```python
from build123d import *

# Parameters (mm, degrees)
SKETCH_1_4_R        = 75
BOSS_EXTRUDE1_DEPTH = 18
SKETCH_1_3_R        = 50
BOSS_EXTRUDE2_DEPTH = 210
BOSS_EXTRUDE3_START = -228
SKETCH_1_4_2_R      = 75
BOSS_EXTRUDE3_DEPTH = 18


with BuildPart() as part:
    # Sketch 1_4 → Boss-Extrude1 (new body)
    with BuildSketch(Plane(origin=(0, 0, 0), x_dir=(0, 0, -1), z_dir=(1, 0, 0))):
        Circle(SKETCH_1_4_R)
    extrude(amount=BOSS_EXTRUDE1_DEPTH)

    # 草图1<3> → Boss-Extrude2 (add)
    with BuildSketch(Plane(origin=(0, 0, 0), x_dir=(0, 0, -1), z_dir=(1, 0, 0))):
        Circle(SKETCH_1_3_R)
    extrude(amount=-BOSS_EXTRUDE2_DEPTH)

    # Sketch 1_4 2 → Boss-Extrude3 (add)
    with BuildSketch(Plane(origin=(0, 0, 0), x_dir=(0, 0, -1), z_dir=(1, 0, 0)).offset(BOSS_EXTRUDE3_START)):
        Circle(SKETCH_1_4_2_R)
    extrude(amount=BOSS_EXTRUDE3_DEPTH)


solid = part.part
```
Here's how the part is built. I have some questions about the finished solid (model axes, mm). A direction names the side the tool comes from. Coordinates: 2 decimals unless noted, no trailing zeros. Order: outer loops, then holes, each group sorted by start corner. A loop starts at its lowest first (then second) coordinate and runs counter-clockwise, first axis right, second up. Notation, with made-up numbers: (-32, -11.75) - (-19, -11.75) arc R20 ccw to (-19, 21.25) - close; hole circle Ø10 at (-1, 51). An arc over 180 degrees is marked (long way). One line per question, with ' | ' between items.
(1) Will these pins go through, and if not, where does the flat tip stop? pin 1 (10 mm diameter, centred on x = -96, z = 37, fed in from +Y); pin 2 (12 mm diameter, centred on x = -123, y = 32, fed in from +Z); pin 3 (10 mm diameter, centred on x = -163, z = 20.5, fed in from +Y).
Report:
pin 1: stops at y = 38.42 | pin 2: stops at z = 42.71 | pin 3: stops at y = 47.54
(2) If we mould it in two halves opening along X, with no side actions, what happens to faces 1 (the flat face through (18, 1, 1)), 2 (the flat face through (-228, 1, 1)), 3 (the cylindrical face through (8.874, 74.362, 9.764)), 4 (the flat face through (-210, -16, -49))? For each: pulls with the +X half, pulls with the -X half, needs draft (parallel to the pull), parting line crosses it, or undercut.
Report:
face 1: pulls with the +X half | face 2: pulls with the -X half | face 3: needs draft | face 4: undercut
(3) If I drill on L1, parallel to X at y = 18, z = -53; L2, parallel to Y at x = -213.5, z = 12; L3, parallel to Y at x = -166, z = 37, over which ranges is the centre line in solid material (lowest first)?
Report:
L1: x = -228 to -210, 0 to 18 | L2: y = -74.03 to 74.03 | L3: y = -33.63 to 33.63
(4) Suppose I cut it at D-D on x = -86. List the corners of the cut face in (y, z) for me.
Report:
outline: circle Ø100 at (0, 0)
(5) Suppose I cut it at A-A on y = 54. List the corners of the cut face in (x, z) for me, and give its area (3 significant figures).
Report:
outline: (-228, -52.05) - (-210, -52.05) - (-210, 52.05) - (-228, 52.05) - close; (0, -52.05) - (18, -52.05) - (18, 52.05) - (0, 52.05) - close | area: 3,750 mm2
(6) For faces 5 (the cylindrical face through (-219.126, 74.362, 9.764)), 6 (the flat face through (0, -16, -49)), which set-ups out of +Z, -Z, +X, -X, +Y, -Y let a thin tool reach every point of the face, with its end or its side?
Report:
face 5: +X, -X | face 6: none
(7) Suppose I cut it at B-B on z = 0. List the corners of the cut face in (x, y) for me.
Report:
outline: (-228, -75) - (-210, -75) - (-210, -50) - (0, -50) - (0, -75) - (18, -75) - (18, 75) - (0, 75) - (0, 50) - (-210, 50) - (-210, 75) - (-228, 75) - close
